from build123d import *

# Parameters (mm, degrees)
SKETCH1_R           = 75
BOSS_EXTRUDE1_DEPTH = 12
SKETCH2_R           = 50
SKETCH2_R_2         = 27.5
BOSS_EXTRUDE2_DEPTH = 28.5
CUT_EXTRUDE1_START  = -18
SKETCH3_R           = 50
SKETCH3_R_2         = 48.675
CUT_EXTRUDE1_DEPTH  = 2.65
CHAMFER1_SIZE       = 2
SKETCH7_R           = 4
CUT_EXTRUDE2_DEPTH  = 110.828275048
SKETCH10_R          = 2.5
CUT_EXTRUDE3_DEPTH  = 7
SKETCH12_R          = 0.5
CUT_EXTRUDE8_DEPTH  = 109.223149095


with BuildPart() as part:
    # Sketch1 → Boss-Extrude1 (new body)
    with BuildSketch(Plane.XY):
        Circle(SKETCH1_R)
    extrude(amount=BOSS_EXTRUDE1_DEPTH)

    # Sketch2 → Boss-Extrude2 (add)
    with BuildSketch(Plane.XY):
        with Locations(Location((0, 0, 0), (0, 0, 180))):
            Circle(SKETCH2_R)
        with Locations(Location((0, 0, 0), (0, 0, 180))):
            Circle(SKETCH2_R_2, mode=Mode.SUBTRACT)
    extrude(amount=BOSS_EXTRUDE2_DEPTH)

    # Sketch3 → Cut-Extrude1 (cut)
    with BuildSketch(Plane(origin=(0, 0, 0), x_dir=(-1, 0, 0), z_dir=(0, 0, -1)).offset(CUT_EXTRUDE1_START)):
        Circle(SKETCH3_R)
        Circle(SKETCH3_R_2, mode=Mode.SUBTRACT)
    extrude(amount=-CUT_EXTRUDE1_DEPTH, mode=Mode.SUBTRACT)

    # Chamfer1
    chamfer1_edges = [part.edges().sort_by_distance(p)[0] for p in [
        (27.5, 0, 28.5),
    ]]
    chamfer(chamfer1_edges, length=CHAMFER1_SIZE)

    # Sketch7 → Cut-Extrude2 (cut, through all)
    with BuildSketch(Plane(origin=(0, 0, 0), x_dir=(-1, 0, 0), z_dir=(0, 0, -1))):
        with Locations((-25.564662216, 63.011491379)):
            Circle(SKETCH7_R)
        with Locations((41.787221156, 53.645392608)):
            Circle(SKETCH7_R)
        with Locations((67.351883372, -9.366098771)):
            Circle(SKETCH7_R)
        with Locations((25.564662216, -63.011491379)):
            Circle(SKETCH7_R)
        with Locations((-41.787221156, -53.645392608)):
            Circle(SKETCH7_R)
        with Locations((-67.351883372, 9.366098771)):
            Circle(SKETCH7_R)
    extrude(amount=-CUT_EXTRUDE2_DEPTH, mode=Mode.SUBTRACT)

    # Sketch10 → Cut-Extrude3 (cut)
    with BuildSketch(Plane(origin=(0, 0, 0), x_dir=(-1, 0, 0), z_dir=(0, 0, -1))):
        with Locations((10.150674704, -25.019268636)):
            Circle(SKETCH10_R)
    extrude(amount=-CUT_EXTRUDE3_DEPTH, mode=Mode.SUBTRACT)

    # Sketch12 → Cut-Extrude8 (cut, through all)
    with BuildSketch(Plane(origin=(0, 0, 7), x_dir=(-1, 0, 0), z_dir=(0, 0, -1))):
        with Locations((10.150674704, -25.019268636)):
            Circle(SKETCH12_R)
    extrude(amount=-CUT_EXTRUDE8_DEPTH, mode=Mode.SUBTRACT)


solid = part.part
Work out the finished part from the listing and answer in its coordinate system (mm). A direction names the side the tool comes from. Round coordinates to 2 decimals unless told otherwise and drop trailing zeros. Write each loop counter-clockwise with the first axis right and the second up, starting at its lowest first coordinate (ties: lowest second). Pieces come first, ordered by that corner, then holes. Notation, with made-up numbers: (-22.75, 18) - (22.25, 18) arc R9 cw to (22.25, 30) - close; hole circle Ø11 at (-40, 40). An arc over 180 degrees is marked (long way). Answer in a Markdown table with one row per item. Add a question column.
1. A cutting plane is placed at A-A, the plane x = -42. Determine the outline of the cut face in (y, z), and give its area (3 significant figures).
2. The mould has two halves that part along X. Classify faces 6 (the cylindrical face through (39.64, -50.27, 5.92)), 7 (the flat face through (49, -16, 12)), 8 (the flat face through (-11, -25, 7)), 9 (the cylindrical face through (-9.764, 74.362, 5.916)): +X half, -X half, draft (parallel to the pull), parting line (faces both ways), or undercut.
3. A cutting plane is placed at B-B, the plane y = 0. Determine the outline of the cut face in (x, z) (3 decimals), and give its area (3 significant figures).
4. Given pin 1 (6 mm diameter, centred on x = -3, z = 20.5, fed in from -Y); pin 2 (12 mm diameter, centred on x = -28, z = 17, fed in from +Y); pin 3 (13 mm diameter, centred on x = 41.79, y = -53.65, fed in from +Z); pin 4 (6.5 mm diameter, centred on x = 67.35, y = 9.37, fed in from +Z), each flat-ended and moving along its own axis, determine where each tip first touches the part or whether it passes through.
5. A cutting plane is placed at D-D, the plane z = 24.25. Determine the outline of the cut face in (x, y).
6. For faces 1 (the cylindrical face through (-47.69, -15.02, 24.52)), 2 (the cylindrical face through (-12.46, -25.98, 3.45)), 3 (the cylindrical face through (29.56, 63.19, 5.92)), 4 (the flat face through (1, -1, 0)), 5 (the cylindrical face through (-46.427, 14.621, 19.306)), determine the directions among +Z, -Z, +X, -X, +Y, -Y from which every point of the face is accessible in a straight line to the end or side of a thin tool.
7. Find the intervals of material crossed by line 1 along Y through (x, z) = (0, 17.75); line 2 along Z through (x, y) = (51, 26); line 3 along Y through (x, z) = (0, 2), in increasing order. Write a range as from..to.
Worked out:
| question | item | result |
|---|---|---|
| 1 | outline | (-62.14, 0) - (49.65, 0) - (49.65, 12) - (27.13, 12) - (27.13, 18) - (24.6, 18) - (24.6, 20.65) - (27.13, 20.65) - (27.13, 28.5) - (-27.13, 28.5) - (-27.13, 20.65) - (-24.6, 20.65) - (-24.6, 18) - (-27.13, 18) - (-27.13, 12) - (-62.14, 12) - close; (57.64, 0) - (62.14, 0) - (62.14, 12) - (57.64, 12) - close |
| 1 | area | 2,280 mm^2 |
| 2 | face 6 | undercut |
| 2 | face 7 | draft |
| 2 | face 8 | undercut |
| 2 | face 9 | parting line |
| 3 | outline | (-75, 0) - (75, 0) - (75, 12) - (50, 12) - (50, 18) - (48.675, 18) - (48.675, 20.65) - (50, 20.65) - (50, 28.5) - (29.5, 28.5) - (27.5, 26.5) - (27.5, 12) - (-27.5, 12) - (-27.5, 26.5) - (-29.5, 28.5) - (-50, 28.5) - (-50, 20.65) - (-48.675, 20.65) - (-48.675, 18) - (-50, 18) - (-50, 12) - (-75, 12) - close |
| 3 | area | 2,530 mm^2 |
| 4 | pin 1 | y = -50 |
| 4 | pin 2 | y = 70.82 |
| 4 | pin 3 | z = 12 |
| 4 | pin 4 | through |
| 5 | outline | circle Ø100 at (0, 0); hole circle Ø55 at (0, 0) |
| 6 | face 1 | +Z |
| 6 | face 2 | -Z |
| 6 | face 3 | +Z, -Z |
| 6 | face 4 | -Z, +X, -X, +Y, -Y |
| 6 | face 5 | none |
| 7 | line 1 | -50..-27.5, 27.5..50 |
| 7 | line 2 | 0..12 |
| 7 | line 3 | -75..75 |
